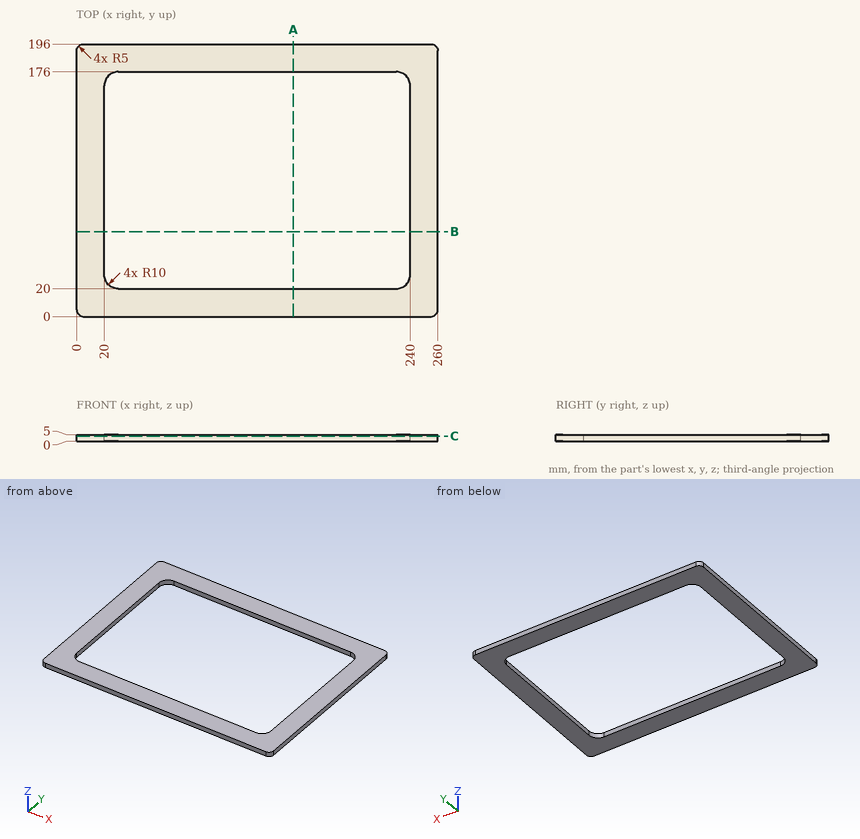
Print and shaded views of the part. All mm, measured from the part's lowest x, y and z. Coordinates: 2 decimals unless noted, no trailing zeros. Write each loop counter-clockwise with the first axis right and the second up, starting at its lowest first coordinate (ties: lowest second). Pieces come first, ordered by that corner, then holes.
(1) Drill centre lines: probe 1 along Y at (x, z) = (121, 1.7); probe 2 along X at (y, z) = (41, 2.7); probe 3 along X at (y, z) = (167, 1.1). Where is each one in solid material? Low to high.
(2) Cut at B-B, the plane y = 61. List the corners of the cut face in (x, z).
(3) Cut at C-C, the plane z = 3.9. List the corners of the cut face in (x, y).
(4) Cut at A-A, the plane x = 156. List the corners of the cut face in (y, z).
Geometry says:
1. probe 1: y = 0 to 20, 176 to 196
1. probe 2: x = 0 to 20, 240 to 260
1. probe 3: x = 0 to 20.05, 239.95 to 260
2. outline: (0, 0) - (20, 0) - (20, 5) - (0, 5) - close; (240, 0) - (260, 0) - (260, 5) - (240, 5) - close
3. outline: (0, 5) arc R5 ccw to (5, 0) - (255, 0) arc R5 ccw to (260, 5) - (260, 191) arc R5 ccw to (255, 196) - (5, 196) arc R5 ccw to (0, 191) - close; hole (20, 30) arc R10 ccw to (30, 20) - (230, 20) arc R10 ccw to (240, 30) - (240, 166) arc R10 ccw to (230, 176) - (30, 176) arc R10 ccw to (20, 166) - close
4. outline: (0, 0) - (20, 0) - (20, 5) - (0, 5) - close; (176, 0) - (196, 0) - (196, 5) - (176, 5) - close
